Build history of the part. All positions in model axes, mm. A direction names the side the tool comes from. Give positions to 0.01 mm unless a question says otherwise; leave off trailing zeros. Order: outer loops, then holes, each group sorted by start corner. A loop starts at its lowest first (then second) coordinate and runs counter-clockwise, first axis right, second up. Notation, with made-up numbers: (46.5, 86.5) -> (75.5, 86.5) arc R30 ccw to (75.5, 116.5) -> close; hole circle Ø10 at (25.5, -36). An arc over 180 degrees is marked (long way). One line per item, written item: value. Start each with the question number.
(1) Probe line 1 (X direction, y = 8.25, z = 5); line 2 (Y direction, x = 69, z = 0); line 3 (Z direction, x = 34, y = 1.5). List the from-to ranges inside material, lowest first.
(2) Which spindle directions (+Z, -Z, +X, -X, +Y, -Y) get a long thin tool onto all of the face, cutting with end or side? Do faces 1 (the cylindrical face through (41.56, 7.81, -1.73)), 2 (the flat face through (9.2, -12.4, 0)), 3 (the flat face through (9.2, 6, -11)), 4 (the flat face through (9.2, 6, 11)). Say none if no direction does.
(3) Saw through at A-A on x = 27. Give the cut face in (y, z), plus the area to 3 significant figures.
(4) Pin check, flat tips, straight feed: pin 1 (2 mm diameter, centred on x = 8, y = -10, fed in from +Z); pin 2 (1 mm diameter, centred on x = 58, y = -4, fed in from +Z); pin 3 (5 mm diameter, centred on x = 42.5, z = -7, fed in from +Y). Stop position of each tip, or through.
```python
from build123d import *

# Parameters (mm, degrees)
EXTRUDE_365_DEPTH = 10
SKETCH_4_W        = 0.8
SKETCH_4_H        = 11.856406461
CHAMFER_2062_SIZE = 1.6
FILLET_2107_R     = 0.6


with BuildPart() as part:
    # 草图1 → Extrude 365 (new body)
    with BuildSketch(Plane(origin=(0, 0, 0), x_dir=(0, 0, -1), z_dir=(1, 0, 0))):
        Polygon((12, 6.92820323), (12, -6.92820323), (0, -13.856406461), (-12, -6.92820323), (-12, 6.92820323), (0, 13.856406461), align=None)
    extrude(amount=EXTRUDE_365_DEPTH)

    # 草图2 → 凸台-旋转1 (revolve)
    with BuildSketch(Plane.XY, mode=Mode.PRIVATE) as revolve_1_sk:
        Polygon((0, 0), (75, 0), (75, 6.268), (75, 8), (7.791693541, 8), (0, 8), align=None)
    revolve(revolve_1_sk.sketch.rotate(Axis((0, 0, 0), (1, 0, 0)), 90), axis=Axis((0, 0, 0), (1, 0, 0)))

    # 草图3 → 切除-旋转1 (revolve, cut)
    with BuildSketch(Plane.XY):
        Polygon((0, 12), (3.958548116, 18.856406461), (3.958548116, 23.856406461), (-10, 23.856406461), (-10, 12), align=None)
    revolve(axis=Axis((0, 0, 0), (1, 0, 0)), mode=Mode.SUBTRACT)

    # 草图5 → 切除-旋转2 (revolve, cut)
    with BuildSketch(Plane.XY):
        Polygon((10, 12), (6.041451884, 18.856406461), (6.041451884, 23.856406461), (16.041451884, 23.856406461), (16.041451884, 12), align=None)
    revolve(axis=Axis((0, 0, 0), (1, 0, 0)), mode=Mode.SUBTRACT)

    # 草图4 → 切除-旋转3 (revolve, cut)
    with BuildSketch(Plane.XY, mode=Mode.PRIVATE) as cut_revolve_3_sk:
        with Locations((9.6, 17.928203231)):
            Rectangle(SKETCH_4_W, SKETCH_4_H)
    revolve(cut_revolve_3_sk.sketch.rotate(Axis((0, 0, 0), (1, 0, 0)), 270), axis=Axis((0, 0, 0), (1, 0, 0)), mode=Mode.SUBTRACT)

    # Chamfer 2062
    chamfer_2062_edges = [part.edges().sort_by_distance(p)[0] for p in [
        (75, 0, -8),
    ]]
    chamfer(chamfer_2062_edges, length=CHAMFER_2062_SIZE)

    # Fillet 2107
    fillet_2107_edges = [part.edges().sort_by_distance(p)[0] for p in [
        (10, 0, -8),
    ]]
    fillet(fillet_2107_edges, radius=FILLET_2107_R)


solid = part.part
```
Results below:
1. line 1: x = 0 to 10
1. line 2: y = -8 to 8
1. line 3: z = -7.86 to 7.86
2. face 1: +X
2. face 2: +X, -Y
2. face 3: -Z, +X, +Y
2. face 4: +Z, +X, +Y
3. outline: circle Ø16 at (0, 0)
3. area: 201 mm²
4. pin 1: stops at z = 8.41
4. pin 2: stops at z = 7.19
4. pin 3: stops at y = 6.61
